Geometry: see drawing. Coordinates: mm, zero at the bounding-box minimum. A direction names the side the tool comes from. Coordinates: 2 decimals unless noted, no trailing zeros. Write each loop counter-clockwise with the first axis right and the second up, starting at its lowest first coordinate (ties: lowest second). Pieces come first, ordered by that corner, then holes. Notation, with made-up numbers: (68, -0.5) - (97, -0.5) arc R25 ccw to (97, 23.5) - close; hole circle Ø7 at (-6.5, -2). An arc over 180 degrees is marked (long way). One line per question, with ' | ' between items. Start each with the question number.
Q1. Cut plane B-B, the plane z = 33. Return loops of the section in (x, y), plus the area to 3 significant figures.
Q2. Cut plane C-C, the plane x = 181.5. Return loops of the section in (y, z).
Q3. Draft query along Z for the marked faces 4, 5 and 6. Return one class per face: +Z half, -Z half, draft (parallel to the pull), parting line (faces both ways), or undercut.
Q4. Access query for the marked faces 1, 2 and 3. Directions: +Z, -Z, +X, -X, +Y, -Y. A direction counts if a zero-diameter tool reaches every point of the face in a straight line with its end or side. Return the directions, or none.
Q5. Cut plane A-A, the plane y = 8.75. Return loops of the section in (x, z).
Q6. Contact query for flat-ended pins moving along their axis: P1, Ø12, axis at x = 73.5, z = 41, coming from the -Y side; P2, Ø0.6, axis at x = 138, y = 25, coming from the -Z side; P3, Ø14.5, axis at x = 98.5, z = 4.5, coming from the +Y side. Output: stop coordinate, or through.
Q7. Line query: line 1 (X direction, y = 5.75, z = 33); line 2 (X direction, y = 3, z = 19); line 3 (Z direction, x = 156, y = 7.5). Output: solid intervals per line, ascending.
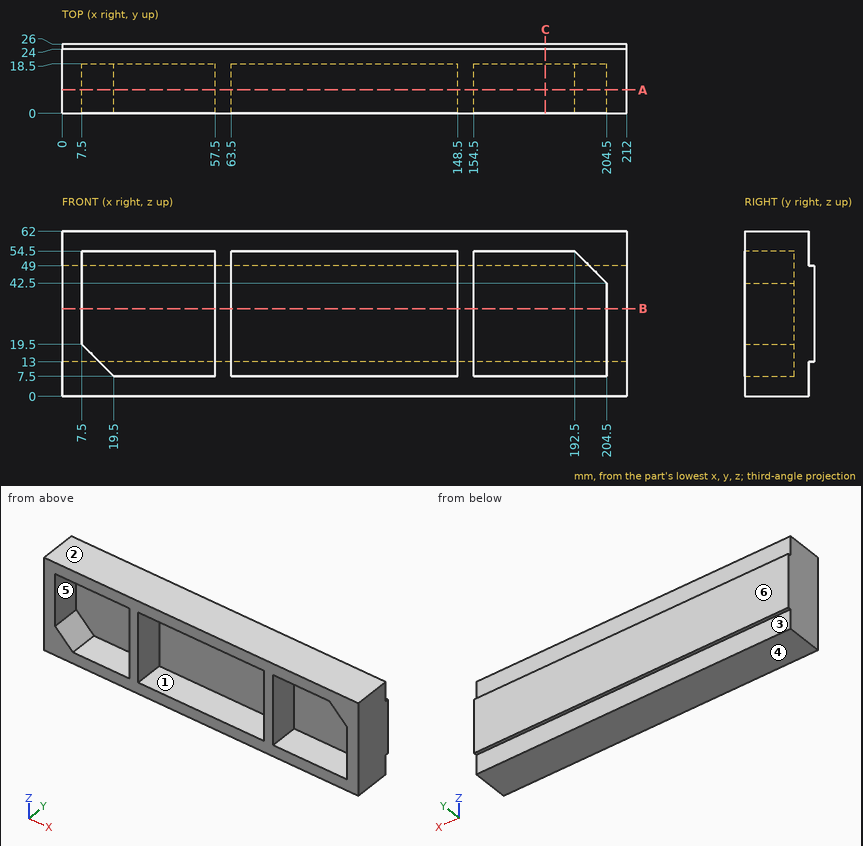
Reply:
1) outline: (0, 0) - (7.5, 0) - (7.5, 18.5) - (57.5, 18.5) - (57.5, 0) - (63.5, 0) - (63.5, 18.5) - (148.5, 18.5) - (148.5, 0) - (154.5, 0) - (154.5, 18.5) - (204.5, 18.5) - (204.5, 0) - (212, 0) - (212, 26) - (0, 26) - close | area: 2,090 mm^2
2) outline: (0, 0) - (24, 0) - (24, 13) - (26, 13) - (26, 49) - (24, 49) - (24, 62) - (0, 62) - (0, 54.5) - (18.5, 54.5) - (18.5, 7.5) - (0, 7.5) - close
3) face 4: -Z half | face 5: undercut | face 6: draft
4) face 1: -Y | face 2: +Z, +X, -X, +Y, -Y | face 3: -Z, +X, -X, +Y
5) outline: (0, 0) - (212, 0) - (212, 62) - (0, 62) - close; hole (7.5, 19.5) - (19.5, 7.5) - (57.5, 7.5) - (57.5, 54.5) - (7.5, 54.5) - close; hole (63.5, 7.5) - (148.5, 7.5) - (148.5, 54.5) - (63.5, 54.5) - close; hole (154.5, 7.5) - (204.5, 7.5) - (204.5, 42.5) - (192.5, 54.5) - (154.5, 54.5) - close
6) P1: stops at y = 18.5 | P2: stops at z = 13 | P3: stops at y = 24
7) line 1: x = 0 to 7.5, 57.5 to 63.5, 148.5 to 154.5, 204.5 to 212 | line 2: x = 0 to 8, 57.5 to 63.5, 148.5 to 154.5, 204.5 to 212 | line 3: z = 0 to 7.5, 54.5 to 62
